Input: dimensioned drawing with shaded views. Units: mm. Origin: part minimum x, y, z. Give positions to 0.01 mm unless a question says otherwise; leave off trailing zeros. Write each loop counter-clockwise with the first axis right and the second up, starting at its lowest first coordinate (ties: lowest second). Pieces come first, ordered by that corner, then holes.
Q1. Section B-B (z = 25.25). Return the cut outline in (x, y).
Q2. Line query: line 1 (Y direction, x = 2.1, z = 27); line 2 (X direction, y = 2.15, z = 3.5); line 3 (Y direction, x = 1.05, z = 9.5). Output: solid intervals per line, ascending.
Q3. Pin query (flat end, axial travel): pin 1 Ø0.6 at (x, z) = (1.5, 25) entering from +Y. Return the tip coordinate at first contact, or that it passes through.
Q4. Section A-A (x = 2). Return the cut outline in (y, z), plus the area to 3 significant figures.
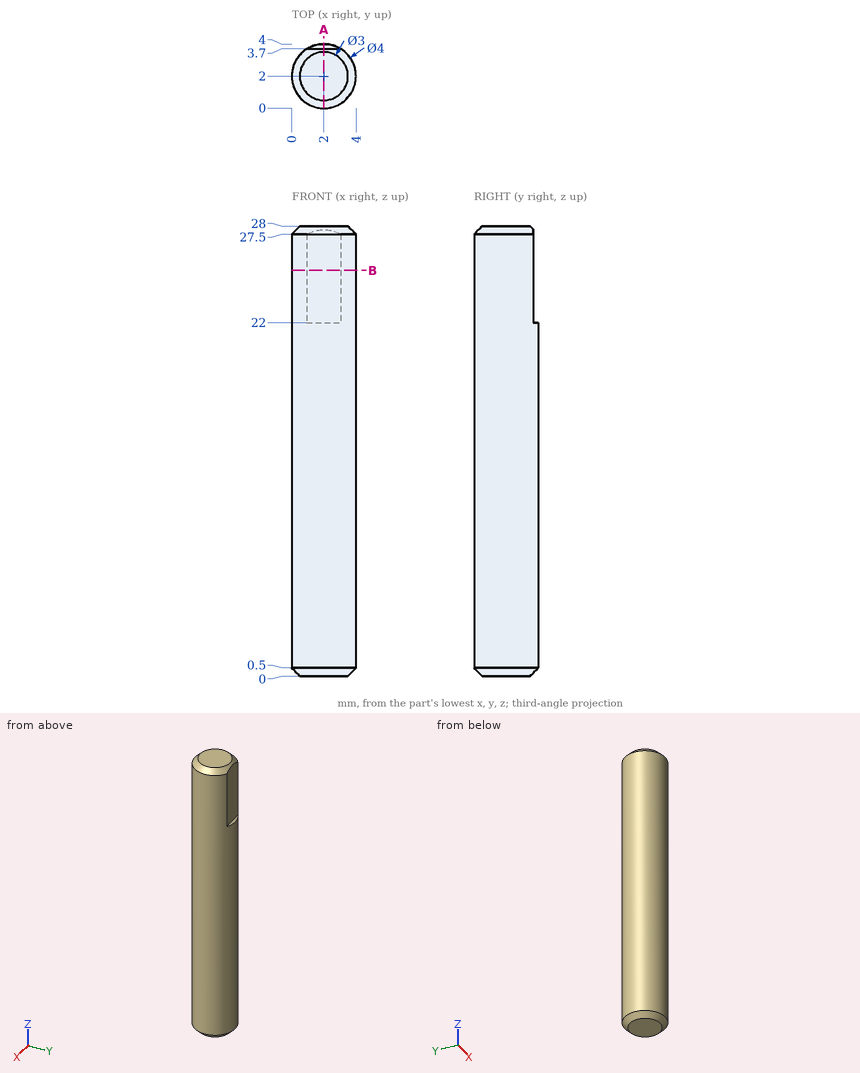
Computed:
1. outline: (0.95, 3.7) arc R2 ccw (long way) to (3.05, 3.7) - close
2. line 1: y = 0 to 3.7
2. line 2: x = 0.01 to 3.99
2. line 3: y = 0.24 to 3.76
3. pin 1: stops at y = 3.7
4. outline: (0, 0.5) - (0.5, 0) - (3.5, 0) - (4, 0.5) - (4, 22) - (3.7, 22) - (3.7, 27.8) - (3.5, 28) - (0.5, 28) - (0, 27.5) - close
4. area: 110 mm2
